from build123d import *

# Parameters (mm, degrees)
BASE_PLATE_DEPTH          = 10
MOUNTING_HOLES_SKETCH_R   = 10
MOUNTING_HOLES_4X_DEPTH   = 10
UPRIGHT_TAB_SKETCH_W      = 10
UPRIGHT_TAB_SKETCH_H      = 120
UPRIGHT_TAB_DEPTH         = 65
TAB_CORNER_FILLET_1_R10_R = 10
TAB_CORNER_FILLET_2_R10_R = 10
TAB_HOLE_SKETCH_R         = 12.5
TAB_HOLE_DEPTH            = 65


with BuildPart() as part:
    # Base Plate Sketch → Base Plate (new body)
    with BuildSketch(Plane(origin=(0, 0, 0), x_dir=(1, 0, 0), z_dir=(0, 1, 0))):
        with BuildLine():
            Line((-130, -87.5), (130, -87.5))
            ThreePointArc((130, -87.5), (144.142135624, -81.642135624), (150, -67.5))
            Line((150, -67.5), (150, 67.5))
            ThreePointArc((150, 67.5), (144.142135624, 81.642135624), (130, 87.5))
            Line((130, 87.5), (-130, 87.5))
            ThreePointArc((-130, 87.5), (-144.142135624, 81.642135624), (-150, 67.5))
            Line((-150, 67.5), (-150, -67.5))
            ThreePointArc((-150, -67.5), (-144.142135624, -81.642135624), (-130, -87.5))
        make_face()
    extrude(amount=BASE_PLATE_DEPTH)

    # Mounting Holes Sketch → Mounting Holes 4x (cut)
    with BuildSketch(Plane(origin=(0, 10, 0), x_dir=(1, 0, 0), z_dir=(0, 1, 0))):
        with Locations(Location((130, 67.5, 0), (0, 0, 270))):
            Circle(MOUNTING_HOLES_SKETCH_R)
        with Locations(Location((130, -67.5, 0), (0, 0, 270))):
            Circle(MOUNTING_HOLES_SKETCH_R)
        with Locations(Location((-130, 67.5, 0), (0, 0, 270))):
            Circle(MOUNTING_HOLES_SKETCH_R)
        with Locations(Location((-130, -67.5, 0), (0, 0, 270))):
            Circle(MOUNTING_HOLES_SKETCH_R)
    extrude(amount=-MOUNTING_HOLES_4X_DEPTH, mode=Mode.SUBTRACT)

    # Upright Tab Sketch → Upright Tab (add)
    with BuildSketch(Plane(origin=(0, 10, 0), x_dir=(1, 0, 0), z_dir=(0, 1, 0))):
        Rectangle(UPRIGHT_TAB_SKETCH_W, UPRIGHT_TAB_SKETCH_H)
    extrude(amount=UPRIGHT_TAB_DEPTH)

    # Tab Corner Fillet 1 R10
    tab_corner_fillet_1_r10_edges = [part.edges().sort_by_distance(p)[0] for p in [
        (0, 75, 60),
    ]]
    fillet(tab_corner_fillet_1_r10_edges, radius=TAB_CORNER_FILLET_1_R10_R)

    # Tab Corner Fillet 2 R10
    tab_corner_fillet_2_r10_edges = [part.edges().sort_by_distance(p)[0] for p in [
        (0, 75, -60),
    ]]
    fillet(tab_corner_fillet_2_r10_edges, radius=TAB_CORNER_FILLET_2_R10_R)

    # Tab Hole Sketch → Tab Hole (cut)
    with BuildSketch(Plane(origin=(5, 0, 0), x_dir=(0, 0, -1), z_dir=(1, 0, 0))):
        with Locations((0, 55)):
            Circle(TAB_HOLE_SKETCH_R)
    extrude(amount=-TAB_HOLE_DEPTH, mode=Mode.SUBTRACT)


solid = part.part
Input: part model. Units: mm. Frame: model coordinates. Give positions to 0.01 mm unless a question says otherwise; leave off trailing zeros. Write each loop counter-clockwise with the first axis right and the second up, starting at its lowest first coordinate (ties: lowest second). Pieces come first, ordered by that corner, then holes.
Q1. First-contact query: P1, Ø19.5, axis at y = 29, z = -16.5, coming from the -X side; P2, Ø3, axis at x = -14.5, z = 50, coming from the +Y side; P3, Ø12, axis at y = 39.5, z = -3, coming from the +X side. Flat tips, straight axial feed; report the tip coordinate or a pass-through.
Q2. Pull-direction query (Y, two-part tool) for faces 1 (the face through (0.07, 67.394, 1.627)), 2 (the face through (2, 5, -87.5)), 3 (the face through (-2, 0, -1)); classes: pulls with the +Y half, pulls with the -Y half, needs draft (parallel to the pull), parting line crosses it, or undercut.
Q3. Material intervals for probe 1 along X at (y, z) = (4, 67); probe 2 along Y at (x, z) = (0, 0); probe 3 along Y at (x, z) = (85, 73), sorted ascending.
Q4. Section B-B, the plane y = 6. Output: boundary loops of the cut face in (x, z).
Q5. Section A-A, the plane z = 0. Output: boundary loops of the cut face in (x, y).
Q6. Section D-D, the plane z = -42. Output: boundary loops of the cut face in (x, y), plus the area to 3 significant figures.
Q7. Section C-C, the plane y = 55. Output: boundary loops of the cut face in (x, z), plus the area to 3 significant figures.
Filled in:
1. P1: stops at x = -5
1. P2: stops at y = 10
1. P3: stops at x = 5
2. face 1: undercut
2. face 2: needs draft
2. face 3: pulls with the -Y half
3. probe 1: x = -150 to -139.99, -120.01 to 120.01, 139.99 to 150
3. probe 2: y = 0 to 42.5, 67.5 to 75
3. probe 3: y = 0 to 10
4. outline: (-150, -67.5) arc R20 ccw to (-130, -87.5) - (130, -87.5) arc R20 ccw to (150, -67.5) - (150, 67.5) arc R20 ccw to (130, 87.5) - (-130, 87.5) arc R20 ccw to (-150, 67.5) - close; hole circle Ø20 at (-130, -67.5); hole circle Ø20 at (-130, 67.5); hole circle Ø20 at (130, -67.5); hole circle Ø20 at (130, 67.5)
5. outline: (-150, 0) - (150, 0) - (150, 10) - (5, 10) - (5, 42.5) - (-5, 42.5) - (-5, 10) - (-150, 10) - close; (-5, 67.5) - (5, 67.5) - (5, 75) - (-5, 75) - close
6. outline: (-150, 0) - (150, 0) - (150, 10) - (5, 10) - (5, 75) - (-5, 75) - (-5, 10) - (-150, 10) - close
6. area: 3,650 mm2
7. outline: (-5, -60) - (5, -60) - (5, -12.5) - (-5, -12.5) - close; (-5, 12.5) - (5, 12.5) - (5, 60) - (-5, 60) - close
7. area: 950 mm2
